Geometry check sheet. Reference: the model listing, model coordinates, mm. A direction names the side the tool comes from. Round coordinates to 2 decimals unless told otherwise and drop trailing zeros. Order: outer loops, then holes, each group sorted by start corner. A loop starts at its lowest first (then second) coordinate and runs counter-clockwise, first axis right, second up. Notation, with made-up numbers: (28.25, 0.25) - (46.25, 0.25) arc R16 cw to (46.25, 31.25) - close; hole circle Ø2 at (80, -15). An arc over 180 degrees is marked (long way). One line per question, with ' | ' between items. Start each with the question number.
Q1. Tool access check on faces 1 (the face through (225, 10, 11)), 2 (the face through (-156.767, 10, -68)), 3 (the face through (-171.767, -4, 1)). Record the directions out of +Z, -Z, +X, -X, +Y, -Y that give a thin tool (end or side, any length) a straight path to the whole face; none if there is none.
Q2. Mould release check, pull along Z, two halves, no side actions. Record for faces 4 (the face through (-192, 5, 60)), 5 (the face through (240.511, 10, 32)), 6 (the face through (-99.7, 9.86, 30.79)): +Z half, -Z half, draft (parallel to the pull), parting line (faces both ways), or undercut.
Q3. Sectioned sample at A-A, the plane z = -40. Enter the section's corners in (x, y), then the cut area to 3 significant figures.
Q4. Sectioned sample at B-B, the plane z = 0. Enter the section's corners in (x, y).
Q5. Sectioned sample at C-C, the plane y = -4. Enter the section's corners in (x, z), then the cut area to 3 significant figures.
Q6. Sectioned sample at D-D, the plane z = 46.5. Enter the section's corners in (x, y), then the cut area to 3 significant figures.
Q7. Gauge pin test, flat ends, axial feed: P1, Ø1, axis at y = -25.5, z = -52, coming from the -X side; P2, Ø18.5, axis at y = 8.5, z = 72, coming from the -X side; P3, Ø22, axis at x = 224.5, y = 14, coming from the +Z side; P4, Ø10, axis at x = -67, y = -8, coming from the +Z side. Record the tip position at first contact, or that the pin passes through.
Q8. Material ranges on line 1 along X through (y, z) = (13.5, -47); line 2 along X through (y, z) = (13, -40); line 3 along X through (y, z) = (-8.5, 47.5), recorded low to high.
```python
from build123d import *

# Parameters (mm, degrees)
SKETCH1_R           = 12.5
SKETCH1_R_2         = 15
BOSS_EXTRUDE1_DEPTH = 20
SKETCH2_R           = 12.5
BOSS_EXTRUDE3_DEPTH = 60


with BuildPart() as part:
    # Sketch1 → Boss-Extrude1 (new body)
    with BuildSketch(Plane(origin=(0, 0, 0), x_dir=(1, 0, 0), z_dir=(0, 1, 0))):
        with BuildLine():
            Line((-156.766665721, -76.687206232), (82.57489949, -76.687206232))
            Line((82.57489949, -76.687206232), (240.511245974, -51.99105161))
            Line((240.511245974, -51.99105161), (240.511245974, -11))
            Line((240.511245974, -11), (208.511245974, -11))
            ThreePointArc((208.511245974, -11), (198.376578208, 0), (208.511245974, 11))
            Line((208.511245974, 11), (240.511245974, 11))
            Line((240.511245974, 11), (240.511245974, 49))
            Line((240.511245974, 49), (82.57489949, 76.687206232))
            Line((82.57489949, 76.687206232), (-156.766665721, 76.687206232))
            Line((-156.766665721, 76.687206232), (-156.766665721, 60))
            Line((-156.766665721, 60), (-171.766665721, 60))
            Line((-171.766665721, 60), (-171.766665721, -60))
            Line((-171.766665721, -60), (-156.766665721, -60))
            Line((-156.766665721, -60), (-156.766665721, -76.687206232))
        make_face()
        with Locations(Location((-108.150428542, 40, 0), (0, 0, 270))):
            Circle(SKETCH1_R, mode=Mode.SUBTRACT)
        with Locations(Location((-108.150428542, -40, 0), (0, 0, 270))):
            Circle(SKETCH1_R, mode=Mode.SUBTRACT)
        with Locations(Location((91.849571458, 40, 0), (0, 0, 270))):
            Circle(SKETCH1_R, mode=Mode.SUBTRACT)
        with Locations(Location((91.849571458, -40, 0), (0, 0, 270))):
            Circle(SKETCH1_R, mode=Mode.SUBTRACT)
        with Locations(Location((151.849571458, 0, 0), (0, 0, 270))):
            Circle(SKETCH1_R_2, mode=Mode.SUBTRACT)
    extrude(amount=BOSS_EXTRUDE1_DEPTH)

    # Sketch2 → Boss-Extrude3 (add, symmetric)
    with BuildSketch(Plane.XY):
        with BuildLine():
            Line((-199.766665721, 20), (-171.766665721, 20))
            Line((-171.766665721, 20), (-171.766665721, -8))
            ThreePointArc((-171.766665721, -8), (-219.565655594, -27.798989873), (-199.766665721, 20))
        make_face()
        with Locations((-199.766665721, -8)):
            Circle(SKETCH2_R, mode=Mode.SUBTRACT)
    extrude(amount=BOSS_EXTRUDE3_DEPTH, both=True)


solid = part.part
```
Determined:
1) face 1: +X, +Y, -Y | face 2: -Z, -X, +Y, -Y | face 3: +Z, -Z, +X, -Y
2) face 4: +Z half | face 5: draft | face 6: undercut
3) outline: (-199.77, 20) arc R28 ccw (long way) to (-171.77, -8) - (-171.77, 0) - (-120.65, 0) - (-120.65, 20) - close; (-95.65, 0) - (79.35, 0) - (79.35, 20) - (-95.65, 20) - close; (104.35, 0) - (240.51, 0) - (240.51, 20) - (104.35, 20) - close; hole circle Ø25 at (-199.77, -8) | area: 9,390 mm2
4) outline: (-199.77, 20) arc R28 ccw (long way) to (-171.77, -8) - (-171.77, 0) - (136.85, 0) - (136.85, 20) - close; (166.85, 0) - (198.38, 0) - (198.38, 20) - (166.85, 20) - close; hole circle Ø25 at (-199.77, -8)
5) outline: (-227.48, -60) - (-211.61, -60) - (-211.61, 60) - (-227.48, 60) - close; (-187.92, -60) - (-171.77, -60) - (-171.77, 60) - (-187.92, 60) - close | area: 3,840 mm2
6) outline: (-199.77, 20) arc R28 ccw (long way) to (-171.77, -8) - (-171.77, 0) - (-118.83, 0) - (-118.83, 20) - close; (-97.47, 0) - (81.17, 0) - (81.17, 20) - (-97.47, 20) - close; (102.53, 0) - (240.51, 0) - (240.51, 20) - (102.53, 20) - close; hole circle Ø25 at (-199.77, -8) | area: 9,530 mm2
7) P1: stops at x = -222.02 | P2: stops at x = -156.77 | P3: stops at z = 56.21 | P4: passes through
8) line 1: x = -217.7 to -118.51, -97.79 to 81.49, 102.21 to 240.51 | line 2: x = -218.29 to -120.65, -95.65 to 79.35, 104.35 to 240.51 | line 3: x = -227.76 to -212.26, -187.28 to -171.77
